```python
from build123d import *

# Parameters (mm, degrees)
UNEQUAL_ANGLE_STEEL_6_3_4_1_DEPTH = 75
M6_CLEARANCE_HOLE1_D              = 6.6
M6_CLEARANCE_HOLE1_DEPTH          = 20
M6_CLEARANCE_HOLE1_TIP            = 1.982840043
CUT_EXTRUDE1_DEPTH                = 106.80170131
CUT_EXTRUDE1_DEPTH_BACK           = 106.80170131
SKETCH8_W                         = 14
SKETCH8_H                         = 16
FILLET1_R                         = 5


with BuildPart() as part:
    # Sketch11 → Unequal Angle Steel 6.3-4(1) (new body)
    with BuildSketch(Plane.YZ):
        with BuildLine():
            Line((63, 0), (0, 0))
            Line((0, 0), (0, -40))
            Line((0, -40), (4.666666667, -40))
            ThreePointArc((4.666666667, -40), (6.316582489, -39.316582489), (7, -37.666666667))
            Line((7, -37.666666667), (7, -14))
            ThreePointArc((7, -14), (9.050252532, -9.050252532), (14, -7))
            Line((14, -7), (60.666666667, -7))
            ThreePointArc((60.666666667, -7), (62.316582489, -6.316582489), (63, -4.666666667))
            Line((63, -4.666666667), (63, 0))
        make_face()
    extrude(amount=UNEQUAL_ANGLE_STEEL_6_3_4_1_DEPTH)

    # M6 Clearance Hole1
    with Locations(Plane.XZ):
        with Locations((15, -28), (60, -28)):
            Hole(M6_CLEARANCE_HOLE1_D / 2, depth=M6_CLEARANCE_HOLE1_DEPTH)
            with Locations((0, 0, -(M6_CLEARANCE_HOLE1_DEPTH + M6_CLEARANCE_HOLE1_TIP / 2))):  # 118° drill point
                Cone(0, M6_CLEARANCE_HOLE1_D / 2, M6_CLEARANCE_HOLE1_TIP, mode=Mode.SUBTRACT)

    # Sketch8 → Cut-Extrude1 (cut, two sides: drawn at the far end of the back side and taken through both)
    with BuildSketch(Plane(origin=(75, 0, 0), x_dir=(0, 0, -1), z_dir=(1, 0, 0)).offset(-CUT_EXTRUDE1_DEPTH_BACK)):
        with Locations((0, 63)):
            Rectangle(SKETCH8_W, SKETCH8_H)
    extrude(amount=CUT_EXTRUDE1_DEPTH + CUT_EXTRUDE1_DEPTH_BACK, mode=Mode.SUBTRACT)

    # Fillet1
    fillet1_edges = [part.edges().sort_by_distance(p)[0] for p in [
        (0, 55, -3.5),
        (75, 55, -3.5),
    ]]
    fillet(fillet1_edges, radius=FILLET1_R)


solid = part.part
```
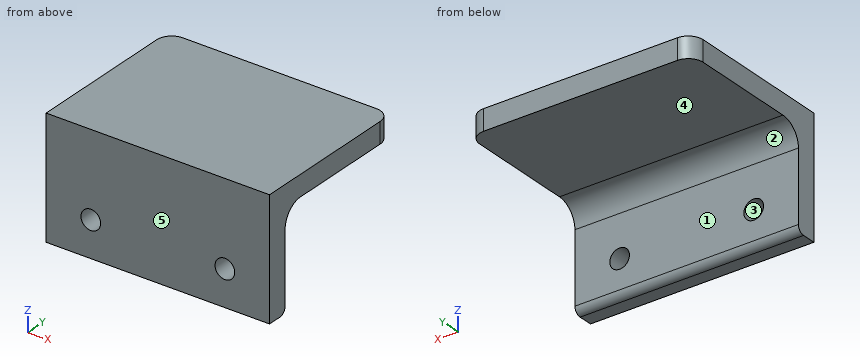
The model under review builds one solid part; all positions refer to its coordinate system, in mm. Face numbers are marked on the shaded views. A direction names the side the tool comes from. Round coordinates to 2 decimals unless told otherwise and drop trailing zeros. Order: outer loops, then holes, each group sorted by start corner. A loop starts at its lowest first (then second) coordinate and runs counter-clockwise, first axis right, second up. Notation, with made-up numbers: (-9.75, 80.5) - (26.25, 80.5) arc R31 ccw to (26.25, 116.5) - close; hole circle Ø7 at (26, -30.5). An arc over 180 degrees is marked (long way). Answer in a Markdown table with one row per item.
(1) Take a section at B-B on x = 60. Write out the cut boundary in (y, z).
Result set:
| item | result |
|---|---|
| outline | (0, -40) - (4.67, -40) arc R2.33 ccw to (7, -37.67) - (7, -31.3) - (0, -31.3) - close; (0, -24.7) - (7, -24.7) - (7, -14) arc R7 cw to (14, -7) - (55, -7) - (55, 0) - (0, 0) - close |
(2) Clearance check with flat-ended pins moving along their axes: P1, Ø1, axis at x = 41.5, y = 27.5, coming from the +Z side; P2, Ø2, axis at x = 54, z = -24.5, coming from the +Y side; P3, Ø20.5, axis at x = 42.5, y = 42.5, coming from the -Z side. State where each tip first meets the part, or that it passes through.
Result set:
| item | result |
|---|---|
| P1 | stops at z = 0 |
| P2 | stops at y = 7 |
| P3 | stops at z = -7 |
(3) Mouldability with a two-part tool opening along Z and no side actions: class the marked faces 1, 2 and 3 as released by +Z, released by -Z, zero draft, split by the parting line, or undercut.
Result set:
| item | result |
|---|---|
| face 1 | zero draft |
| face 2 | released by -Z |
| face 3 | undercut |
(4) For line 1 (Z direction, x = 60, y = 3); line 2 (Z direction, x = 65.5, y = 35.5); line 3 (Y direction, x = 50, z = -31), list the stretches that pass through material, from the lowest coordinate up. Write a range as from..to.
Result set:
| item | result |
|---|---|
| line 1 | z = -40..-31.3, -24.7..0 |
| line 2 | z = -7..0 |
| line 3 | y = 0..7 |
(5) Take a section at A-A on z = -28. Write out the cut boundary in (x, y).
Result set:
| item | result |
|---|---|
| outline | (0, 0) - (11.7, 0) - (11.7, 7) - (0, 7) - close; (18.3, 0) - (56.7, 0) - (56.7, 7) - (18.3, 7) - close; (63.3, 0) - (75, 0) - (75, 7) - (63.3, 7) - close |
(6) Machinability: for the marked faces 4 and 5, which of the approach directions +Z, -Z, +X, -X, +Y, -Y give a long, thin tool a straight path to every point of the face, cutting with its end or side? Answer none if there is none.
Result set:
| item | result |
|---|---|
| face 4 | -Z, +X, -X, +Y |
| face 5 | +Z, -Z, +X, -X, -Y |
(7) Take a section at D-D on y = 35. Write out the cut boundary in (x, z).
Result set:
| item | result |
|---|---|
| outline | (0, -7) - (75, -7) - (75, 0) - (0, 0) - close |
(8) Take a section at C-C on x = 49.5. Write out the cut boundary in (y, z).
Result set:
| item | result |
|---|---|
| outline | (0, -40) - (4.67, -40) arc R2.33 ccw to (7, -37.67) - (7, -14) arc R7 cw to (14, -7) - (55, -7) - (55, 0) - (0, 0) - close |
